Design review of the part built by this model. Coordinates are the model's own, in mm. Face numbers are marked on the shaded views. Round coordinates to 2 decimals unless told otherwise and drop trailing zeros. Order: outer loops, then holes, each group sorted by start corner. A loop starts at its lowest first (then second) coordinate and runs counter-clockwise, first axis right, second up.
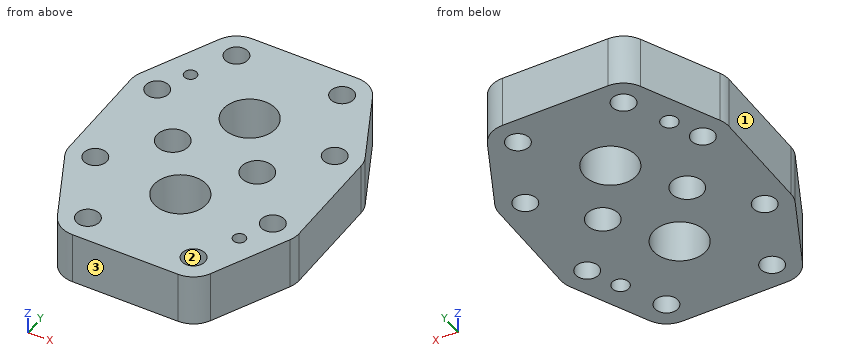
from build123d import *

# Parameters (mm, degrees)
BOSS_EXTRUDE2_DEPTH = 25
SKETCH_19_5_R       = 5.5
SKETCH_19_5_R_2     = 12.5
SKETCH_19_5_R_3     = 7.5
CUT_EXTRUDE1_DEPTH  = 95.082410683
SKETCH_19_6_R       = 3
CUT_EXTRUDE5_DEPTH  = 95.082410683
SKETCH_19_7_2_R     = 4
CUT_EXTRUDE7_DEPTH  = 12


with BuildPart() as part:
    # Sketch 19_7 → Boss-Extrude2 (new body)
    with BuildSketch(Plane.XY):
        with BuildLine():
            Line((54.5, -25), (54.5, 25))
            ThreePointArc((54.5, 25), (54.181915896, 27.801950234), (53.243851982, 30.461299534))
            Line((53.243851982, 30.461299534), (36.243851982, 65.461299534))
            ThreePointArc((36.243851982, 65.461299534), (31.632637327, 70.595193348), (25, 72.5))
            Line((25, 72.5), (-25, 72.5))
            ThreePointArc((-25, 72.5), (-31.632637327, 70.595193348), (-36.243851982, 65.461299534))
            Line((-36.243851982, 65.461299534), (-53.243851982, 30.461299534))
            ThreePointArc((-53.243851982, 30.461299534), (-54.181915896, 27.801950234), (-54.5, 25))
            Line((-54.5, 25), (-54.5, -25))
            ThreePointArc((-54.5, -25), (-54.181915896, -27.801950234), (-53.243851982, -30.461299534))
            Line((-53.243851982, -30.461299534), (-36.243851982, -65.461299534))
            ThreePointArc((-36.243851982, -65.461299534), (-31.632637327, -70.595193348), (-25, -72.5))
            Line((-25, -72.5), (25, -72.5))
            ThreePointArc((25, -72.5), (31.632637327, -70.595193348), (36.243851982, -65.461299534))
            Line((36.243851982, -65.461299534), (53.243851982, -30.461299534))
            ThreePointArc((53.243851982, -30.461299534), (54.181915896, -27.801950234), (54.5, -25))
        make_face()
    extrude(amount=BOSS_EXTRUDE2_DEPTH)

    # 草图19<5> → Cut-Extrude1 (cut, through all)
    with BuildSketch(Plane.XY):
        with Locations((-25, 60)):
            Circle(SKETCH_19_5_R)
        with Locations((-42, 25)):
            Circle(SKETCH_19_5_R)
        with Locations((-42, -25)):
            Circle(SKETCH_19_5_R)
        with Locations((0, -28)):
            Circle(SKETCH_19_5_R_2)
        with Locations((20, 0)):
            Circle(SKETCH_19_5_R_3)
        with Locations((-20, 0)):
            Circle(SKETCH_19_5_R_3)
        with Locations((0, 28)):
            Circle(SKETCH_19_5_R_2)
        with Locations((-25, -60)):
            Circle(SKETCH_19_5_R)
    cut_extrude1 = extrude(amount=CUT_EXTRUDE1_DEPTH, mode=Mode.SUBTRACT)

    # Mirror1: Cut-Extrude1 across plane
    add(cut_extrude1.mirror(Plane(origin=(0, 0, 0), x_dir=(0, 0, 1), z_dir=(1, 0, 0))), mode=Mode.SUBTRACT)

    # 草图19<6> → Cut-Extrude5 (cut, through all)
    with BuildSketch(Plane.XY):
        with Locations((35, -40)):
            Circle(SKETCH_19_6_R)
        with Locations((-35, 40)):
            Circle(SKETCH_19_6_R)
    extrude(amount=CUT_EXTRUDE5_DEPTH, mode=Mode.SUBTRACT)

    # Sketch 19_7 2 → Cut-Extrude7 (cut)
    with BuildSketch(Plane.XY):
        with Locations((-35, 40)):
            Circle(SKETCH_19_7_2_R)
        with Locations((35, -40)):
            Circle(SKETCH_19_7_2_R)
    extrude(amount=CUT_EXTRUDE7_DEPTH, mode=Mode.SUBTRACT)


solid = part.part
1) To check wall thickness, follow line 1 along X through (y, z) = (-18, 22); line 2 along Y through (x, z) = (42, 8.5); line 3 along X through (y, z) = (-39, 8.5). State the ranges of each line that lie inside material, in increasing order.
Results:
line 1: x = -54.5 to -7.5, 7.5 to 54.5
line 2: y = -53.61 to -30.5, -19.5 to 19.5, 30.5 to 53.61
line 3: x = -49.1 to -5.94, 5.94 to 31.13, 38.87 to 49.1
2) Take a section at C-C on z = 20.5. State how many separate pieces and enclosed holes the cut face has, plus the area to 3 significant figures.
Results:
separate pieces: 1
enclosed holes: 14
area: 11,700 mm2
3) The part is to be moulded in two halves that separate along X. For the marked faces 1, 2 and 3, say which applies: released by +X, released by -X, zero draft, split by the parting line, or undercut.
Results:
face 1: released by -X
face 2: undercut
face 3: zero draft
4) Take a section at B-B on y = 0. Give the boundary of the cut face in (x, z).
Results:
outline: (-54.5, 0) - (-27.5, 0) - (-27.5, 25) - (-54.5, 25) - close; (-12.5, 0) - (12.5, 0) - (12.5, 25) - (-12.5, 25) - close; (27.5, 0) - (54.5, 0) - (54.5, 25) - (27.5, 25) - close
5) Take a section at D-D on y = -28. Give the boundary of the cut face in (x, z).
Results:
outline: (-54.13, 0) - (-46.61, 0) - (-46.61, 25) - (-54.13, 25) - close; (-37.39, 0) - (-12.5, 0) - (-12.5, 25) - (-37.39, 25) - close; (12.5, 0) - (37.39, 0) - (37.39, 25) - (12.5, 25) - close; (46.61, 0) - (54.13, 0) - (54.13, 25) - (46.61, 25) - close
6) Take a section at A-A on x = 0. Give the boundary of the cut face in (y, z).
Results:
outline: (-72.5, 0) - (-40.5, 0) - (-40.5, 25) - (-72.5, 25) - close; (-15.5, 0) - (15.5, 0) - (15.5, 25) - (-15.5, 25) - close; (40.5, 0) - (72.5, 0) - (72.5, 25) - (40.5, 25) - close
7) Clearance check with flat-ended pins moving along their axes: P1, Ø9, axis at x = 20, y = 0, coming from the +Z side; P2, Ø1, axis at y = -43, z = 9.5, coming from the -X side; P3, Ø3, axis at y = -31.5, z = 16.5, coming from the -X side; P4, Ø6.5, axis at x = -35, y = 40, coming from the -Z side. State where each tip first meets the part, or that it passes through.
Results:
P1: passes through
P2: stops at x = -47.4
P3: stops at x = -53.46
P4: stops at z = 12
